from build123d import *


with BuildPart() as part:
    # Sketch1 → Revolve1 (revolve)
    with BuildSketch(Plane.XY, mode=Mode.PRIVATE) as revolve1_sk:
        Polygon((-2.75, -2.226189364), (-9, -2.226189364), (-9, 1.773810636), (-14, 1.773810636), (-14, -0.226189364), (-16, -0.226189364), (-16, 3.773810636), (-6.214101615, 3.773810636), (-2.75, 1.773810636), align=None)
    revolve(revolve1_sk.sketch.rotate(Axis((0, 9.90888507, 0), (0, -1, 0)), 270), axis=Axis((0, 9.90888507, 0), (0, -1, 0)))


solid = part.part
Here's how the part is built. I have some questions about the finished solid (model axes, mm). A direction names the side the tool comes from. Give positions to 0.01 mm unless a question says otherwise; leave off trailing zeros. Order: outer loops, then holes, each group sorted by start corner. A loop starts at its lowest first (then second) coordinate and runs counter-clockwise, first axis right, second up. Notation, with made-up numbers: (9.25, -34.5) -> (53.25, -34.5) arc R23 cw to (53.25, -14.5) -> close; hole circle Ø8 at (46, 4.5). An arc over 180 degrees is marked (long way). One line per item, written item: value. Start each with the question number.
1. I need wall thicknesses on probe 1 along X at (y, z) = (-1.35, 0); probe 2 along Z at (x, y) = (-5.5, 1.65); probe 3 along Z at (x, y) = (-3.5, 0.5). Which ranges of each line are inside material? Lowest first, please. Write a range as from..to.
2. Imagine slicing it at A-A, the plane x = 0. List the corners of the cut face in (y, z) for me.
3. Imagine slicing it at B-B, the plane z = 0. List the corners of the cut face in (x, y) for me, plus the area to 3 significant figures.
4. Imagine slicing it at D-D, the plane z = 7. List the corners of the cut face in (x, y) for me.
5. We'd pull the mould along Z, two halves only. Please class faces 3 (the face through (-2.1, -2.226, 2.1)), 4 (the face through (2.685, -0.254, -0.596)), 5 (the face through (15.62, 1.8, -3.47)), 6 (the face through (13.67, 0.76, -3.03)): released by +Z, released by -Z, zero draft, split by the parting line, or undercut.
6. Imagine slicing it at C-C, the plane y = 1.2. List the corners of the cut face in (x, z) for me, plus the area to 3 significant figures.
7. Will these pins go through, and if not, where does the flat tip stop? pin 1 Ø3 at (x, y) = (3, 0) entering from -Z; pin 2 Ø1.5 at (y, z) = (1, -2.5) entering from +X; pin 3 Ø6.5 at (x, z) = (0, 0) entering from +Y.
8. For faces 1 (the face through (2.85, 1.87, -0.63)), 2 (the face through (14.15, -0.226, 0.07)), which set-ups out of +Z, -Z, +X, -X, +Y, -Y let a thin tool reach every point of the face, with its end or its side?
Values follow:
1. probe 1: x = -9..-2.75, 2.75..9
1. probe 2: z = -15.02..-12.87, -7.12..7.12, 12.87..15.02
1. probe 3: z = -15.61..-13.56, -8.29..8.29, 13.56..15.61
2. outline: (-2.23, -9) -> (1.77, -9) -> (1.77, -14) -> (-0.23, -14) -> (-0.23, -16) -> (3.77, -16) -> (3.77, -6.21) -> (1.77, -2.75) -> (-2.23, -2.75) -> close; (-2.23, 2.75) -> (1.77, 2.75) -> (3.77, 6.21) -> (3.77, 16) -> (-0.23, 16) -> (-0.23, 14) -> (1.77, 14) -> (1.77, 9) -> (-2.23, 9) -> close
3. outline: (-16, -0.23) -> (-14, -0.23) -> (-14, 1.77) -> (-9, 1.77) -> (-9, -2.23) -> (-2.75, -2.23) -> (-2.75, 1.77) -> (-6.21, 3.77) -> (-16, 3.77) -> close; (2.75, -2.23) -> (9, -2.23) -> (9, 1.77) -> (14, 1.77) -> (14, -0.23) -> (16, -0.23) -> (16, 3.77) -> (6.21, 3.77) -> (2.75, 1.77) -> close
3. area: 104 mm2
4. outline: (-14.39, -0.23) -> (-12.12, -0.23) -> (-12.12, 1.77) -> (-5.66, 1.77) -> (-5.66, -2.23) -> (5.66, -2.23) -> (5.66, 1.77) -> (12.12, 1.77) -> (12.12, -0.23) -> (14.39, -0.23) -> (14.39, 3.77) -> (-14.39, 3.77) -> close
5. face 3: zero draft
5. face 4: undercut
5. face 5: split by the parting line
5. face 6: undercut
6. outline: circle Ø32 at (0, 0); circle Ø18 at (0, 0); hole circle Ø28 at (0, 0); hole circle Ø5.5 at (0, 0)
6. area: 419 mm2
7. pin 1: stops at z = -15.93
7. pin 2: stops at x = 15.9
7. pin 3: stops at y = 2.06
8. face 1: +Y
8. face 2: -Y
